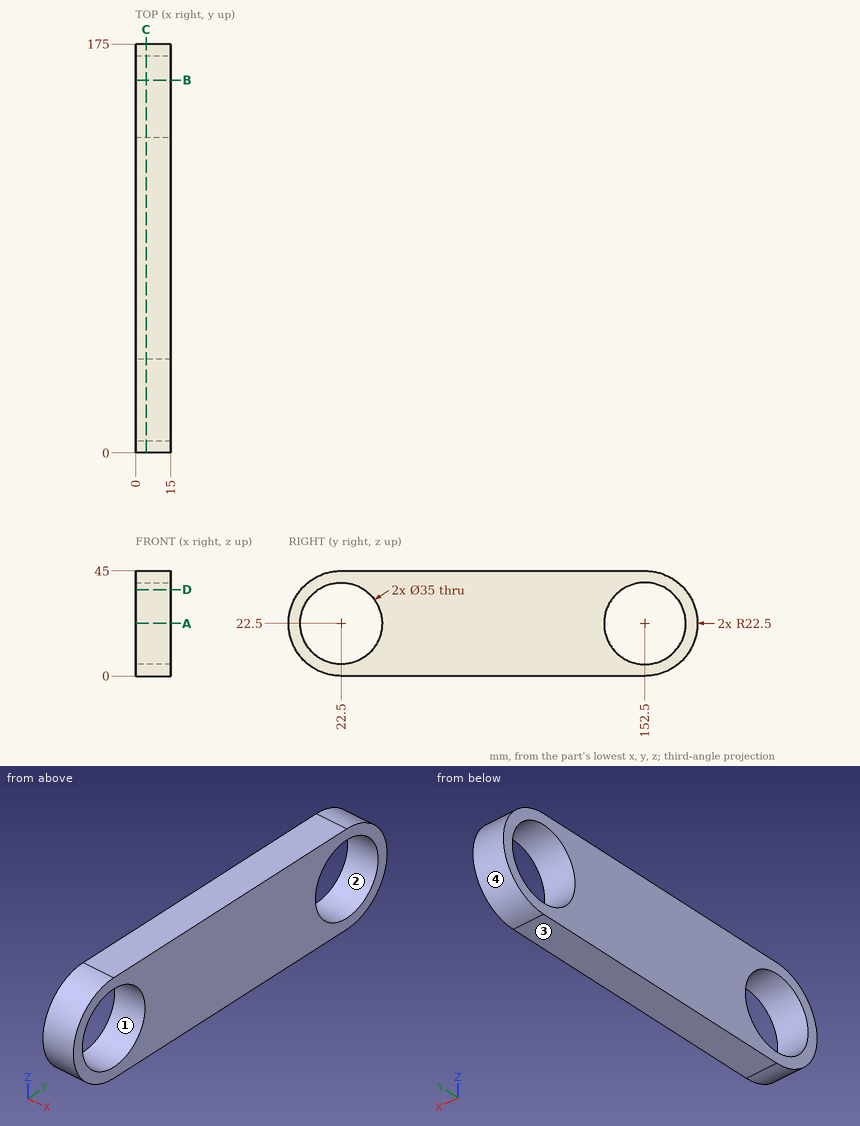
Verification items for this drawing (mm, ordinates from the low corner). Give positions to 0.01 mm unless a question says otherwise; leave off trailing zeros. Loops run counter-clockwise (first coordinate to the right, second up) from the corner with the lowest first, then second, coordinate; pieces in that order, holes last. Notation, with made-up numbers: (-32, 1.25) - (-28, 1.25) arc R15 ccw to (-28, 26.25) - close; hole circle Ø2 at (67, 84.25). An arc over 180 degrees is marked (long way). Write item = value, one per line. Start each with the question number.
Q1. Cross-section at C-C, the plane x = 4.5. Enter the section's corners in (y, z), and give its area (3 significant figures).
Q2. Thickness scan on line 1 (Y direction, x = 4, z = 22.5); line 2 (Y direction, x = 4.25, z = 20.5); line 3 (Z direction, x = 13.75, y = 137.5). Record the ranges inside material, lowest first.
Q3. Cross-section at B-B, the plane y = 159.5. Enter the section's corners in (x, z), and give its area (3 significant figures).
Q4. Mould release check, pull along Z, two halves, no side actions. Record for the marked faces 1, 2, 3 and 4: released by +Z, released by -Z, zero draft, split by the parting line, or undercut.
Q5. Cross-section at A-A, the plane z = 22.5. Enter the section's corners in (x, y), and give its area (4 significant figures).
Q6. Cross-section at D-D, the plane z = 37. Enter the section's corners in (x, y).
Q7. Depth check by flat-ended pin: P1, Ø1, axis at x = 11.5, z = 32, coming from the -Y side; P2, Ø4, axis at x = 4.5, z = 5, coming from the -Y side; P3, Ø2, axis at x = 10, z = 5, coming from the +Y side. Enter the tip coordinate at first touch or a pass-through.
Answer key:
q1.outline = (22.5, 0) - (152.5, 0) arc R22.5 ccw to (152.5, 45) - (22.5, 45) arc R22.5 ccw to start; hole circle Ø35 at (22.5, 22.5); hole circle Ø35 at (152.5, 22.5)
q1.area = 5,520 mm^2
q2.line_1 = 0 to 5, 40 to 135, 170 to 175
q2.line_2 = 0.09 to 5.11, 39.89 to 135.11, 169.89 to 174.91
q2.line_3 = 0 to 13.49, 31.51 to 45
q3.outline = (0, 1.12) - (15, 1.12) - (15, 6.46) - (0, 6.46) - close; (0, 38.54) - (15, 38.54) - (15, 43.88) - (0, 43.88) - close
q3.area = 160 mm^2
q4.face_1 = undercut
q4.face_2 = undercut
q4.face_3 = released by -Z
q4.face_4 = split by the parting line
q5.outline = (0, 0) - (15, 0) - (15, 5) - (0, 5) - close; (0, 40) - (15, 40) - (15, 135) - (0, 135) - close; (0, 170) - (15, 170) - (15, 175) - (0, 175) - close
q5.area = 1,575 mm^2
q6.outline = (0, 5.3) - (15, 5.3) - (15, 12.7) - (0, 12.7) - close; (0, 32.3) - (15, 32.3) - (15, 142.7) - (0, 142.7) - close; (0, 162.3) - (15, 162.3) - (15, 169.7) - (0, 169.7) - close
q7.P1 = 1.88
q7.P2 = 6.19
q7.P3 = 167.8
